Geometry: final body of the model. Coordinates: model frame, mm. A direction names the side the tool comes from. Give positions to 0.01 mm unless a question says otherwise; leave off trailing zeros. Loops run counter-clockwise (first coordinate to the right, second up) from the corner with the lowest first, then second, coordinate; pieces in that order, holes last. Notation, with made-up numbers: (-37, 84) - (-21, 84) arc R28 ccw to (-21, 121) - close; hole circle Ø10 at (51.25, 71.5). An arc over 180 degrees is marked (long way). Use CSV: the item, a comma, the result in double quotes. Start each with the question number.
```python
from build123d import *

# Parameters (mm, degrees)
BRACKET_BODY_DEPTH      = 30
BOSS_ROUNDING_SKETCH_R  = 9.95
BOSS_ROUNDING_CUT_DEPTH = 60
BORE_CUT_DEPTH          = 60


with BuildPart() as part:
    # Bracket Profile Sketch → Bracket Body (new, symmetric)
    with BuildSketch(Plane(origin=(0, 0, 0), x_dir=(0, 0, -1), z_dir=(1, 0, 0))):
        Polygon((0, 0), (40, 0), (40, 10), (20, 10), (20, 40), (0, 40), align=None)
    extrude(amount=BRACKET_BODY_DEPTH, both=True)

    # Boss Rounding Sketch → Boss Rounding Cut (cut)
    with BuildSketch(Plane(origin=(0, 0, -20), x_dir=(-1, 0, 0), z_dir=(0, 0, -1))):
        with Locations(Location((-10, 20, 0), (0, 0, 90))):
            Circle(BOSS_ROUNDING_SKETCH_R)
    extrude(amount=-BOSS_ROUNDING_CUT_DEPTH, mode=Mode.SUBTRACT)

    # Bore Sketch → Bore Cut (cut)
    with BuildSketch(Plane(origin=(0, 0, -20), x_dir=(-1, 0, 0), z_dir=(0, 0, -1))):
        with BuildLine():
            ThreePointArc((-30, 20), (-24.142135624, 34.142135624), (-10, 40))
            Line((-10, 40), (-30, 40))
            Line((-30, 40), (-30, 20))
        make_face()
        with BuildLine():
            ThreePointArc((-10, 40), (4.142135624, 34.142135624), (10, 20))
            Line((10, 20), (20, 20))
            ThreePointArc((20, 20), (27.071067812, 17.071067812), (30, 10))
            Line((30, 10), (30, 40))
            Line((30, 40), (-10, 40))
        make_face()
    extrude(amount=-BORE_CUT_DEPTH, mode=Mode.SUBTRACT)


solid = part.part
```
Item 1: Reachability of faces 5 (the flat face through (0, 25, -20)), 6 (the flat face through (-15, 20, -10)), 7 (the flat face through (-30, 5, -20)) from +Z, -Z, +X, -X, +Y, -Y: full face, straight path, thin tool, end or side. Return the list, or none.
Item 2: Mould query, pull axis Y, two halves, no side actions, for faces 1 (the flat face through (0, 0, -20)), 2 (the cylindrical face through (19.865, 18.705, -10.14)), 3 (the flat face through (0, 16, 0)), 4 (the flat face through (0, 10, -30)). Classes: pulls with the +Y half, pulls with the -Y half, needs draft (parallel to the pull), parting line crosses it, or undercut.
Item 3: Ray query, probe 1 along Y at (x, z) = (-18.5, -21); probe 2 along X at (y, z) = (23.5, -6.5); probe 3 along Z at (x, y) = (-1.5, 20.5). Return the intervals inside material, ascending.
Item 4: Section D-D (y = 14). Output: boundary loops of the cut face in (x, z).
Item 5: Section C-C (x = -12). Output: boundary loops of the cut face in (y, z).
Item 6: Section A-A (z = -17.5). Output: boundary loops of the cut face in (x, y).
Item 7: Section B-B (y = 27.5). Output: boundary loops of the cut face in (x, z).
Item 8: Pin query (flat end, axial travel): pin 1 Ø5 at (x, z) = (-14, -9.5) entering from +Y; pin 2 Ø2 at (x, z) = (22, -5.5) entering from -Y; pin 3 Ø9 at (x, y) = (-3, 22.5) entering from -Z; pin 4 Ø6 at (x, z) = (-2, -33) entering from +Y. Return the tip coordinate at first contact, or that it passes through.
Outcome:
1,face 5,"-Z, +X, -X, +Y"
1,face 6,"+Z, -Z, -X, +Y"
1,face 7,"+Z, -Z, -X, +Y, -Y"
2,face 1,"pulls with the -Y half"
2,face 2,"undercut"
2,face 3,"needs draft"
2,face 4,"pulls with the +Y half"
3,probe 1,"y = 0 to 10"
3,probe 2,"x = -9.69 to 0.69, 19.31 to 29.69"
3,probe 3,"z = -20 to 0"
4,outline,"(-29.17, -20) - (2.06, -20) - (2.06, 0) - (-29.17, 0) - close; (17.94, -20) - (30, -20) - (30, 0) - (17.94, 0) - close"
5,outline,"(0, -40) - (10, -40) - (10, -20) - (20, -20) - (20, 0) - (0, 0) - close"
6,outline,"(-30, 0) - (30, 0) - (30, 20) arc R20 ccw to (-10, 20) - (-20, 20) arc R10 ccw to (-30, 10) - close; hole circle Ø19.9 at (10, 20)"
7,outline,"(-8.54, -20) - (3.46, -20) - (3.46, 0) - (-8.54, 0) - close; (16.54, -20) - (28.54, -20) - (28.54, 0) - (16.54, 0) - close"
8,pin 1,"stops at y = 20"
8,pin 2,"stops at y = 0"
8,pin 3,"stops at z = -20"
8,pin 4,"stops at y = 10"
